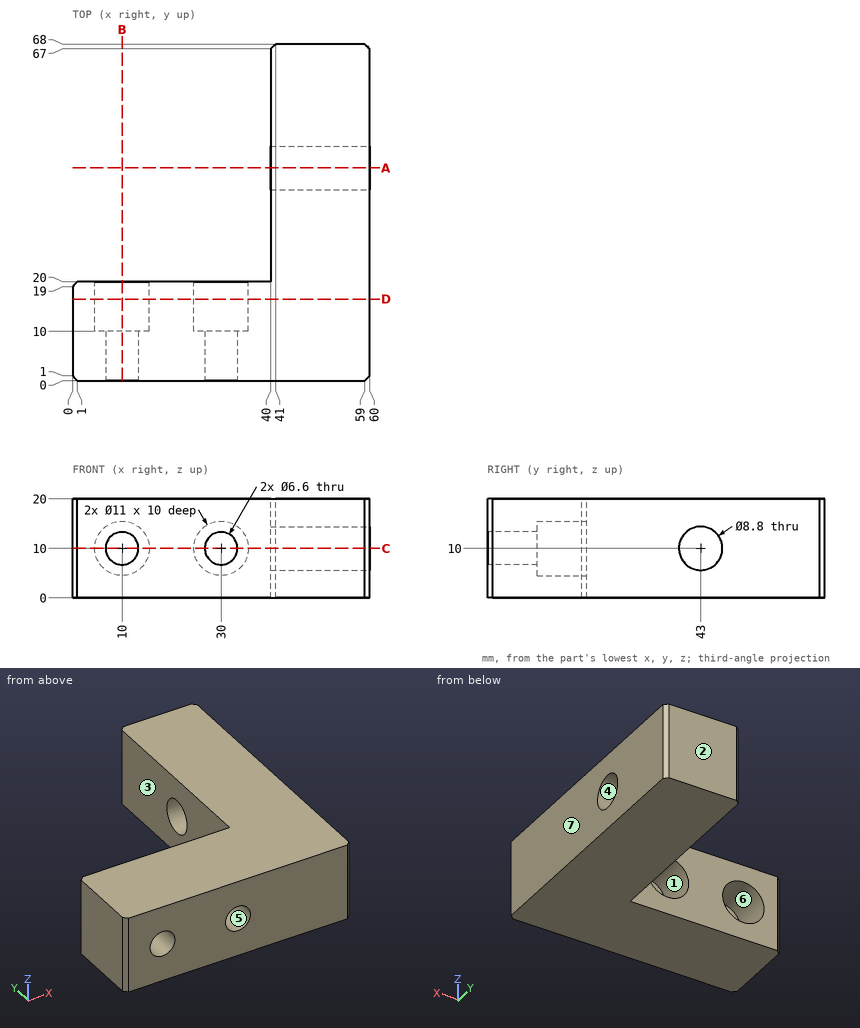
Input: dimensioned drawing with shaded views. Units: mm. Origin: part minimum x, y, z. A direction names the side the tool comes from. Give positions to 0.01 mm unless a question says otherwise; leave off trailing zeros. Write each loop counter-clockwise with the first axis right and the second up, starting at its lowest first coordinate (ties: lowest second). Pieces come first, ordered by that corner, then holes. Notation, with made-up numbers: M 81,21.25 L 133,21.25 A14 ccw 133,46.25 Z; hole C 18,19 d6. An arc over 180 degrees is marked long. Write item = value, one per line. Start each with the question number.
1) Draft query along X for the marked faces 4, 5, 6 and 7. Return one class per face: +X half, -X half, draft (parallel to the pull), parting line (faces both ways), or undercut.
2) First-contact query: pin 1 Ø6 at (x, z) = (20, 7) entering from +Y; pin 2 Ø3.5 at (x, z) = (29.5, 12.5) entering from +Y; pin 3 Ø1 at (y, z) = (38, 10.5) entering from -X; pin 4 Ø6 at (x, z) = (30, 10) entering from +Y. Flat tips, straight axial feed; report the tip coordinate or a pass-through.
3) Reachability of the marked faces 1, 2 and 3 from +Z, -Z, +X, -X, +Y, -Y: full face, straight path, thin tool, end or side. Return the list, or none.
4) Material intervals for line 1 along X through (y, z) = (5.75, 10); line 2 along Z through (x, y) = (10, 6.75); line 3 along X through (y, z) = (18.5, 8.5), sorted ascending. Write a range as [from, to].
5) Cut plane C-C on z = 10. Count the separate pieces of the cut face and the enclosed holes in it, then the cut area to 3 significant figures.
6) Cut plane A-A on y = 43. Return the cut outline in (x, z), then the cut area to 3 significant figures.
7) Cut plane B-B on x = 10. Return the cut outline in (y, z).
8) Cut plane D-D on y = 16.5. Return the cut outline in (x, z).
Solved:
q1.face_4 = draft
q1.face_5 = undercut
q1.face_6 = undercut
q1.face_7 = +X half
q2.pin_1 = 20
q2.pin_2 = 10
q2.pin_3 = 40
q2.pin_4 = through
q3.face_1 = +Y
q3.face_2 = +Z, -Z, +X, -X, +Y
q3.face_3 = +Z, -Z, -X, +Y
q4.line_1 = [0, 6.7], [13.3, 26.7], [33.3, 60]
q4.line_2 = [0, 6.7], [13.3, 20]
q4.line_3 = [0, 4.71], [15.29, 24.71], [35.29, 60]
q5.separate_pieces = 4
q5.enclosed_holes = 0
q5.area = 1,630 mm2
q6.outline = M 40,0 L 60,0 L 60,5.6 L 40,5.6 Z; M 40,14.4 L 60,14.4 L 60,20 L 40,20 Z
q6.area = 224 mm2
q7.outline = M 0,0 L 20,0 L 20,4.5 L 10,4.5 L 10,6.7 L 0,6.7 Z; M 0,13.3 L 10,13.3 L 10,15.5 L 20,15.5 L 20,20 L 0,20 Z
q8.outline = M 0,0 L 60,0 L 60,20 L 0,20 Z; hole C 10,10 d11; hole C 30,10 d11
